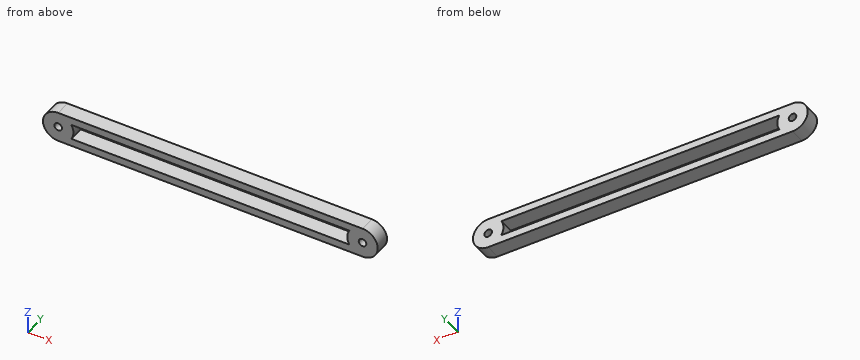
```python
from build123d import *

# Parameters (mm, degrees)
SKETCH1_W           = 400
SKETCH1_H           = 40
BOSS_EXTRUDE1_DEPTH = 20
SKETCH2_W           = 380
SKETCH2_H           = 20
CUT_EXTRUDE1_DEPTH  = 202.990098767
SKETCH4_R           = 20
BOSS_EXTRUDE2_DEPTH = 20
SKETCH6_R           = 5
CUT_EXTRUDE2_DEPTH  = 222.810730128


with BuildPart() as part:
    # Sketch1 → Boss-Extrude1 (new body)
    with BuildSketch(Plane(origin=(0, 0, 0), x_dir=(1, 0, 0), z_dir=(0, 1, 0))):
        Rectangle(SKETCH1_W, SKETCH1_H)
    extrude(amount=BOSS_EXTRUDE1_DEPTH)

    # Sketch2 → Cut-Extrude1 (cut, through all)
    with BuildSketch(Plane(origin=(0, 20, 0), x_dir=(1, 0, 0), z_dir=(0, 1, 0))):
        Rectangle(SKETCH2_W, SKETCH2_H)
    extrude(amount=-CUT_EXTRUDE1_DEPTH, mode=Mode.SUBTRACT)

    # Sketch4 → Boss-Extrude2 (add)
    with BuildSketch(Plane(origin=(0, 20, 0), x_dir=(1, 0, 0), z_dir=(0, 1, 0))):
        with Locations((200, 0)):
            Circle(SKETCH4_R)
        with Locations((-200, 0)):
            Circle(SKETCH4_R)
    extrude(amount=-BOSS_EXTRUDE2_DEPTH)

    # Sketch6 → Cut-Extrude2 (cut, through all)
    with BuildSketch(Plane(origin=(0, 20, 0), x_dir=(1, 0, 0), z_dir=(0, 1, 0))):
        with Locations(Location((200, 0, 0), (0, 0, 270))):
            Circle(SKETCH6_R)
        with Locations(Location((-200, 0, 0), (0, 0, 90))):
            Circle(SKETCH6_R)
    extrude(amount=-CUT_EXTRUDE2_DEPTH, mode=Mode.SUBTRACT)


solid = part.part
```
For this review, take the finished solid that the model builds, in its own axes (mm). Round coordinates to 2 decimals unless told otherwise and drop trailing zeros. Write each loop counter-clockwise with the first axis right and the second up, starting at its lowest first coordinate (ties: lowest second). Pieces come first, ordered by that corner, then holes. Notation, with made-up numbers: (68, 72) - (105, 72) arc R17 cw to (105, 99) - close; hole circle Ø9 at (-12, -1.75). An arc over 180 degrees is marked (long way). Write each question's results on one line, items separated by ' | '.
Item 1: Take a section at C-C on x = -8.5. State the section outline as (y, z) points, then the cut area to 3 significant figures.
Calculated:
outline: (0, -20) - (20, -20) - (20, -10) - (0, -10) - close; (0, 10) - (20, 10) - (20, 20) - (0, 20) - close | area: 400 mm^2
Item 2: To check wall thickness, follow line 1 along X through (y, z) = (5.5, 0); line 2 along Z through (x, y) = (-200, 6.25); line 3 along Z through (x, y) = (159, 14.75). State the ranges of each line that lie inside material, in increasing order. Write a range as from..to.
Calculated:
line 1: x = -220..-205, -195..-180, 180..195, 205..220 | line 2: z = -20..-5, 5..20 | line 3: z = -20..-10, 10..20
Item 3: For pin 1 (8 mm diameter, centred on x = -200, z = 0, fed in from +Y); pin 2 (4 mm diameter, centred on y = 6.5, z = -11, fed in from -X); pin 3 (1 mm diameter, centred on y = 9.5, z = -4, fed in from -X); pin 4 (11.5 mm diameter, centred on x = 200, z = 0, fed in from +Y), all flat-tipped, find the tip position at first contact; note any pin that passes through.
Calculated:
pin 1: passes through | pin 2: stops at x = -217.86 | pin 3: stops at x = -219.69 | pin 4: stops at y = 20
Item 4: Take a section at A-A on y = 15.75. State the section outline as (x, z) points, then the cut area to 3 significant figures.
Calculated:
outline: (-200, -20) - (200, -20) arc R20 ccw to (200, 20) - (-200, 20) arc R20 ccw to start; hole circle Ø10 at (-200, 0); hole (-182.68, -10) - (182.68, -10) arc R20 cw to (182.68, 10) - (-182.68, 10) arc R20 cw to start; hole circle Ø10 at (200, 0) | area: 9,860 mm^2
Item 5: Take a section at B-B on z = 0. State the section outline as (x, y) points.
Calculated:
outline: (-220, 0) - (-205, 0) - (-205, 20) - (-220, 20) - close; (-195, 0) - (-180, 0) - (-180, 20) - (-195, 20) - close; (180, 0) - (195, 0) - (195, 20) - (180, 20) - close; (205, 0) - (220, 0) - (220, 20) - (205, 20) - close
